```python
from build123d import *

# Parameters (mm, degrees)
BOSS_EXTRUDE1_DEPTH = 40
CUT_EXTRUDE1_DEPTH  = 20
SKETCH3_R           = 5
CUT_EXTRUDE2_DEPTH  = 70


with BuildPart() as part:
    # Sketch1 → Boss-Extrude1 (new body)
    with BuildSketch(Plane(origin=(0, 0, 0), x_dir=(1, 0, 0), z_dir=(0, 1, 0))):
        with BuildLine():
            Line((0, 0), (0, -40))
            Line((0, -40), (-32.916811342, -30.326541582))
            ThreePointArc((-32.916811342, -30.326541582), (-40.645313725, -20), (-32.916811342, -9.673458418))
            Line((-32.916811342, -9.673458418), (0, 0))
        make_face()
    extrude(amount=BOSS_EXTRUDE1_DEPTH)

    # Sketch2 → Cut-Extrude1 (cut)
    with BuildSketch(Plane(origin=(0, 10, 0), x_dir=(-1, 0, 0), z_dir=(0, -1, 0))):
        with BuildLine():
            Line((5.381519546, -1.581499041), (5.381519546, -38.418500959))
            Line((5.381519546, -38.418500959), (32.916811342, -30.326541582))
            ThreePointArc((32.916811342, -30.326541582), (40.645313725, -20), (32.916811342, -9.673458418))
            Line((32.916811342, -9.673458418), (5.381519546, -1.581499041))
        make_face()
    extrude(amount=-CUT_EXTRUDE1_DEPTH, mode=Mode.SUBTRACT)

    # Sketch3 → Cut-Extrude2 (cut, symmetric)
    with BuildSketch(Plane(origin=(0, 10, 0), x_dir=(-1, 0, 0), z_dir=(0, -1, 0))):
        with Locations(Location((29.882089371, -20, 0), (0, 0, 90))):
            Circle(SKETCH3_R)
    extrude(amount=CUT_EXTRUDE2_DEPTH, both=True, mode=Mode.SUBTRACT)


solid = part.part
```
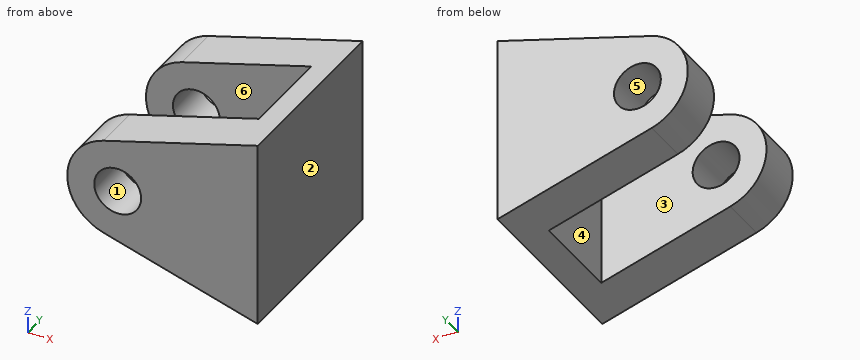
For this review, take the finished solid that the model builds, in its own axes (mm). Face numbers are marked on the shaded views. A direction names the side the tool comes from. Coordinates: 2 decimals unless noted, no trailing zeros. Order: outer loops, then holes, each group sorted by start corner. A loop starts at its lowest first (then second) coordinate and runs counter-clockwise, first axis right, second up. Notation, with made-up numbers: (83, 72.25) -> (129, 72.25) arc R20 ccw to (129, 99.25) -> close; hole circle Ø10 at (23.5, 38.25). An arc over 180 degrees is marked (long way). Use CSV: the item, a comma, the result in double quotes. Start each with the question number.
Item 1: For the marked faces 5 and 6, list the 3-axis set-ups (+Z, -Z, +X, -X, +Y, -Y) from which the entire face can be reached by the end or side of a thin tool; tool diameter is ignored.
Item 2: We need section B-B, the plane x = -35.5. Give the boundary of the cut face in (y, z).
Item 3: Insertion check: pin 1 (1 mm diameter, centred on x = -25, y = 7.5, fed in from +Z); pin 2 (10 mm diameter, centred on y = 16.5, z = 16, fed in from -X). Each pin has a flat end and moves straight along its axis. Give the tip position at first contact, or say it passes through.
Item 4: Draft analysis for pull direction X (two halves, no side actions). For the marked faces 1, 2, 3 and 4, state which applies: pulls with the +X half, pulls with the -X half, needs draft (parallel to the pull), parting line crosses it, or undercut.
Item 5: We need section A-A, the plane z = 20. Give the boundary of the cut face in (x, y), then the cut area to 3 significant figures.
Item 6: We need section D-D, the plane y = 15. Give the boundary of the cut face in (x, z), then the cut area to 3 significant figures.
Item 7: We need section C-C, the plane z = 11.5. Give the boundary of the cut face in (x, y).
Item 8: Wall thickness on probe 1 along Y at (x, z) = (-18, 6); probe 2 along X at (y, z) = (11.5, 10); probe 3 along Z at (x, y) = (-27.5, 36): over which ranges is each line inside the solid? List them lowest first.
Derived:
1,face 5,"+Y, -Y"
1,face 6,"+Z, -Z, -X"
2,outline,"(0, 10.82) -> (10, 10.82) -> (10, 29.18) -> (0, 29.18) -> close; (30, 10.82) -> (40, 10.82) -> (40, 29.18) -> (30, 29.18) -> close"
3,pin 1,"stops at z = 32.8"
3,pin 2,"stops at x = -5.38"
4,face 1,"undercut"
4,face 2,"pulls with the +X half"
4,face 3,"needs draft"
4,face 4,"pulls with the -X half"
5,outline,"(-40.65, 0) -> (-34.88, 0) -> (-34.88, 10) -> (-40.65, 10) -> close; (-40.65, 30) -> (-34.88, 30) -> (-34.88, 40) -> (-40.65, 40) -> close; (-24.88, 0) -> (0, 0) -> (0, 40) -> (-24.88, 40) -> (-24.88, 30) -> (-5.38, 30) -> (-5.38, 10) -> (-24.88, 10) -> close"
5,area,"721 mm^2"
6,outline,"(-5.38, 1.58) -> (0, 0) -> (0, 40) -> (-5.38, 38.42) -> close"
6,area,"207 mm^2"
7,outline,"(-36.48, 0) -> (0, 0) -> (0, 40) -> (-36.48, 40) -> (-36.48, 30) -> (-5.38, 30) -> (-5.38, 10) -> (-36.48, 10) -> close"
8,probe 1,"y = 0 to 10, 30 to 40"
8,probe 2,"x = -5.38 to 0"
8,probe 3,"z = 8.08 to 15.6, 24.4 to 31.92"
